Geometry check sheet. Reference: the model listing, model coordinates, mm. Face numbers are marked on the shaded views. A direction names the side the tool comes from. Round coordinates to 2 decimals unless told otherwise and drop trailing zeros. Order: outer loops, then holes, each group sorted by start corner. A loop starts at its lowest first (then second) coordinate and runs counter-clockwise, first axis right, second up. Notation, with made-up numbers: (29, 34) - (69, 34) arc R27 ccw to (69, 52) - close; hole circle Ø3 at (87.25, -22). An arc over 180 degrees is marked (long way). Write each question's results on one line, items separated by ' | '.
```python
from build123d import *

# Parameters (mm, degrees)
SKETCH1_R           = 58.5
BOSS_EXTRUDE1_DEPTH = 70
SKETCH2_R           = 30
BOSS_EXTRUDE2_DEPTH = 260
BOSS_EXTRUDE4_DEPTH = 28
SKETCH7_R           = 17.5
BOSS_EXTRUDE6_DEPTH = 60
SKETCH8_R           = 10
CUT_EXTRUDE1_DEPTH  = 320.360689612


with BuildPart() as part:
    # Sketch1 → Boss-Extrude1 (new body)
    with BuildSketch(Plane.XY):
        Circle(SKETCH1_R)
    extrude(amount=BOSS_EXTRUDE1_DEPTH)

    # Sketch2 → Boss-Extrude2 (add)
    with BuildSketch(Plane(origin=(0, 0, 0), x_dir=(1, 0, 0), z_dir=(0, 1, 0))):
        with Locations(Location((0, -35, 0), (0, 0, 90))):
            Circle(SKETCH2_R)
    extrude(amount=BOSS_EXTRUDE2_DEPTH)

    # Sketch4 → Boss-Extrude4 (add)
    with BuildSketch(Plane(origin=(0, 260, 0), x_dir=(1, 0, 0), z_dir=(0, 1, 0))):
        with BuildLine():
            Line((0, -65), (45, -65))
            Line((45, -65), (45, -5))
            Line((45, -5), (0, -5))
            ThreePointArc((0, -5), (-30, -35), (0, -65))
        make_face()
    extrude(amount=BOSS_EXTRUDE4_DEPTH)

    # Sketch7 → Boss-Extrude6 (add)
    with BuildSketch(Plane.XY.offset(70)):
        Circle(SKETCH7_R)
    extrude(amount=BOSS_EXTRUDE6_DEPTH)

    # Sketch8 → Cut-Extrude1 (cut, through all)
    with BuildSketch(Plane(origin=(0, 0, 5), x_dir=(-1, 0, 0), z_dir=(0, 0, -1))):
        with Locations((-30, 274)):
            Circle(SKETCH8_R)
    extrude(amount=-CUT_EXTRUDE1_DEPTH, mode=Mode.SUBTRACT)


solid = part.part
```
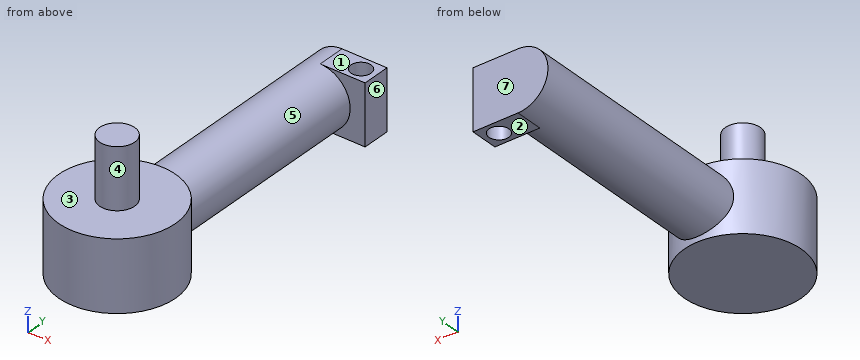
(1) Access from +Z, -Z, +X, -X, +Y, -Y to the whole of each face (thin tool, end or side, straight path). Record for the marked faces 1, 2 and 3.
Answers follow:
face 1: +Z, +X, -X, +Y | face 2: -Z, +X, -X, +Y | face 3: +Z
(2) Section check C-C (y = 0). Record the cut outline in (x, z), then the cut area to 3 significant figures.
Answers follow:
outline: (-58.5, 0) - (58.5, 0) - (58.5, 70) - (17.5, 70) - (17.5, 130) - (-17.5, 130) - (-17.5, 70) - (-58.5, 70) - close | area: 10,300 mm²
(3) Section check A-A (y = 274). Record the cut outline in (x, z).
Answers follow:
outline: (0, 5) - (20, 5) - (20, 65) - (0, 65) arc R30 ccw to start; (40, 5) - (45, 5) - (45, 65) - (40, 65) - close
(4) Draft check along Y on the marked faces 4, 5, 6 and 7. Enter one of: released by +Y, released by -Y, zero draft, split by the parting line, or undercut.
Answers follow:
face 4: split by the parting line | face 5: undercut | face 6: zero draft | face 7: released by +Y
(5) Material ranges on line 1 (Y direction, x = 30, z = 24); line 2 (Y direction, x = 38, z = 41); line 3 (Z direction, x = 28, y = 12), recorded low to high.
Answers follow:
line 1: -50.22 to 50.22, 260 to 264, 284 to 288 | line 2: -44.48 to 44.48, 260 to 268, 280 to 288 | line 3: 0 to 70
(6) Section check D-D (x = -5.5). Record the cut outline in (y, z), then the cut area to 3 significant figures.
Answers follow:
outline: (-58.24, 0) - (58.24, 0) - (58.24, 5.51) - (288, 5.51) - (288, 64.49) - (58.24, 64.49) - (58.24, 70) - (16.61, 70) - (16.61, 130) - (-16.61, 130) - (-16.61, 70) - (-58.24, 70) - close | area: 23,700 mm²
(7) Section check B-B (z = 35). Record the cut outline in (x, y), then the cut area to 3 significant figures.
Answers follow:
outline: (-30, 50.22) arc R58.5 ccw (long way) to (30, 50.22) - (30, 260) - (45, 260) - (45, 288) - (-30, 288) - close; hole circle Ø20 at (30, 274) | area: 24,800 mm²
(8) Depth check by flat-ended pin: pin 1 Ø2 at (x, y) = (16.5, 245.5) entering from +Z; pin 2 Ø14 at (x, y) = (20, 268) entering from +Z; pin 3 Ø13.5 at (x, z) = (20.5, 35.5) entering from -Y. Enter the tip coordinate at first touch or a pass-through.
Answers follow:
pin 1: z = 60.69 | pin 2: z = 65 | pin 3: y = -56.86
